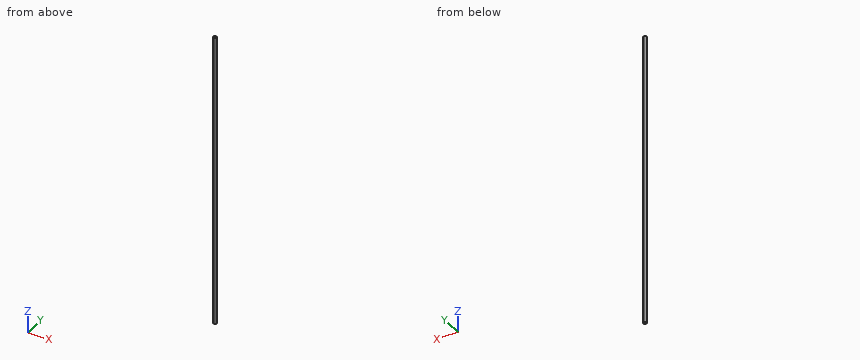
```python
from build123d import *

# Parameters (mm, degrees)
EXTRUDE_1_DEPTH = 900


with BuildPart() as part:
    # 草图1 → 拉伸1 (new body)
    with BuildSketch(Plane.XY):
        with BuildLine():
            Line((-1.661470687, 4.25), (1.661470687, 4.25))
            ThreePointArc((1.661470687, 4.25), (3.001099397, 3.934286669), (4.058769011, 3.053596614))
            ThreePointArc((4.058769011, 3.053596614), (5.079178887, 0), (4.058769011, -3.053596614))
            ThreePointArc((4.058769011, -3.053596614), (3.001099397, -3.934286669), (1.661470687, -4.25))
            Line((1.661470687, -4.25), (-1.661470687, -4.25))
            ThreePointArc((-1.661470687, -4.25), (-3.001099397, -3.934286669), (-4.058769011, -3.053596614))
            ThreePointArc((-4.058769011, -3.053596614), (-5.079178887, 0), (-4.058769011, 3.053596614))
            ThreePointArc((-4.058769011, 3.053596614), (-3.001099397, 3.934286669), (-1.661470687, 4.25))
        make_face()
    extrude(amount=EXTRUDE_1_DEPTH)


solid = part.part
```
Model file for the job. Use its own axes, mm. Round coordinates to 2 decimals unless told otherwise and drop trailing zeros. Loops run counter-clockwise (first coordinate to the right, second up) from the corner with the lowest first, then second, coordinate; pieces in that order, holes last. Notation, with made-up numbers: M 23,46.5 L 59,46.5 A17 ccw 59,54.5 Z; hole C -27.5,36.25 d6. An arc over 180 degrees is marked long. Put each result on its own line as item: value. Start each with the question number.
Item 1: Cut at B-B (y = 1.75). List the corners of the cut face in (x, z).
Item 2: Drill centre lines: line 1 along X through (y, z) = (3.25, 354); line 2 along X through (y, z) = (3, 293); line 3 along Y through (x, z) = (-1.75, 602). Where is each one in solid material? Low to high.
Item 3: Cut at A-A (z = 343.5). List the corners of the cut face in (x, y), then the cut area to 3 significant figures.
Item 4: Drop flat-ended pins along their axis: P1, Ø1, axis at y = 2.5, z = 207, coming from the +X side; P2, Ø1, axis at y = -2, z = 357.5, coming from the +X side; P3, Ø2, axis at y = -1.5, z = 630, coming from the +X side. Give the stop position or say it passes through.
Answer block:
1. outline: M -4.77,0 L 4.77,0 L 4.77,900 L -4.77,900 Z
2. line 1: -3.9 to 3.9
2. line 2: -4.1 to 4.1
2. line 3: -4.25 to 4.25
3. outline: M -4.06,-3.05 A3 ccw -1.66,-4.25 L 1.66,-4.25 A3 ccw 4.06,-3.05 A5.08 ccw 4.06,3.05 A3 ccw 1.66,4.25 L -1.66,4.25 A3 ccw -4.06,3.05 A5.08 ccw Z
3. area: 74.0 mm2
4. P1: x = 4.67
4. P2: x = 4.85
4. P3: x = 5.05
